Read the model definition and answer for the solid it produces. Units are mm, in the model's axes. A direction names the side the tool comes from. Round coordinates to 2 decimals unless told otherwise and drop trailing zeros. Loops run counter-clockwise (first coordinate to the right, second up) from the corner with the lowest first, then second, coordinate; pieces in that order, holes last. Notation, with made-up numbers: (21.5, -23.75) -> (80.5, -23.75) arc R20 cw to (80.5, 7.25) -> close; hole circle Ø7 at (89, -2.75). An arc over 180 degrees is marked (long way). Put each result on its own line as item: value.
from build123d import *

# Parameters (mm, degrees)
CBORE_FOR_M3_HEX_HEAD_BOLT1_D           = 3.5
CBORE_FOR_M3_HEX_HEAD_BOLT1_CBORE_D     = 6
CBORE_FOR_M3_HEX_HEAD_BOLT1_CBORE_DEPTH = 3.5
CHAMFER1_SIZE                           = 0.5


with BuildPart() as part:
    # Sketch1 → Revolve1 (revolve)
    with BuildSketch(Plane.XY, mode=Mode.PRIVATE) as revolve1_sk:
        Polygon((8, 0), (25, 0), (25, 5.5), (11, 5.5), (11, 7), (8, 7), align=None)
    revolve(revolve1_sk.sketch.rotate(Axis((0, 21.458333333, 0), (0, -1, 0)), 90), axis=Axis((0, 21.458333333, 0), (0, -1, 0)))

    # CBORE for M3 Hex Head Bolt1 (through all)
    with Locations(Plane(origin=(-20, 5.5, 0), x_dir=(0, 0, 1), z_dir=(0, 1, 0))):
        with Locations((0, 0), (0, 40)):
            CounterBoreHole(CBORE_FOR_M3_HEX_HEAD_BOLT1_D / 2, CBORE_FOR_M3_HEX_HEAD_BOLT1_CBORE_D / 2, CBORE_FOR_M3_HEX_HEAD_BOLT1_CBORE_DEPTH)

    # Chamfer1
    chamfer1_edges = [part.edges().sort_by_distance(p)[0] for p in [
        (0, 0, -25),
        (0, 0, -8),
        (0, 7, -8),
        (0, 7, -11),
        (0, 5.5, -25),
    ]]
    chamfer(chamfer1_edges, length=CHAMFER1_SIZE)


solid = part.part
Item 1: Flat-ended cylindrical pins translate along their axes: pin 1 Ø5.5 at (x, z) = (20, 0) entering from +Y; pin 2 Ø3 at (y, z) = (1, 4.5) entering from +X; pin 3 Ø2 at (y, z) = (4.5, -13.5) entering from +X. Find the tip coordinate at first contact, or state that the pin passes through.
Derived:
pin 1: stops at y = 2
pin 2: stops at x = 24.82
pin 3: stops at x = 21.65
Item 2: The part is cut by section B-B (z = 0). State how many separate pieces and enclosed holes the cut face has, then the cut area to 3 significant figures.
Derived:
separate pieces: 4
enclosed holes: 0
area: 139 mm^2
Item 3: Find the intervals of material crossed by line 1 along X through (y, z) = (3.15, 0); line 2 along X through (y, z) = (1.1, 0); line 3 along Y through (x, z) = (-8, 15), in increasing order.
Derived:
line 1: x = -25 to -23, -17 to -8, 8 to 17, 23 to 25
line 2: x = -25 to -21.75, -18.25 to -8, 8 to 18.25, 21.75 to 25
line 3: y = 0 to 5.5
Item 4: Which of the six approach directions +Z, -Z, +X, -X, +Y, -Y give full straight-line access (tool end or side, diameter ignored) to faces 4 (the cylindrical face through (7.81, 3.46, -1.73)), 5 (the cylindrical face through (10.74, 6.01, -2.38))?
Derived:
face 4: +Y, -Y
face 5: +Y
Item 5: For a pull along Z with two mould halves and no side action, classify faces 1 (the flat face through (0, 0, -11)), 2 (the cylindrical face through (-7.509, 2.782, 23.846)), 3 (the flat face through (-22, 2, 0)) as pulls with the +Z half, pulls with the -Z half, needs draft (parallel to the pull), parting line crosses it, or undercut.
Derived:
face 1: needs draft
face 2: parting line crosses it
face 3: undercut
Item 6: The part is cut by section A-A (x = 0). Determine the outline of the cut face in (y, z).
Derived:
outline: (0, -24.5) -> (0.5, -25) -> (5, -25) -> (5.5, -24.5) -> (5.5, -11) -> (6.5, -11) -> (7, -10.5) -> (7, -8.5) -> (6.5, -8) -> (0.5, -8) -> (0, -8.5) -> close; (0, 8.5) -> (0.5, 8) -> (6.5, 8) -> (7, 8.5) -> (7, 10.5) -> (6.5, 11) -> (5.5, 11) -> (5.5, 24.5) -> (5, 25) -> (0.5, 25) -> (0, 24.5) -> close
